Design review of the part built by this model. Coordinates are the model's own, in mm. Face numbers are marked on the shaded views. A direction names the side the tool comes from. Give positions to 0.01 mm unless a question says otherwise; leave off trailing zeros. Order: outer loops, then holes, each group sorted by start corner. A loop starts at its lowest first (then second) coordinate and runs counter-clockwise, first axis right, second up. Notation, with made-up numbers: (14, 11) - (48, 11) arc R22 ccw to (48, 32) - close; hole circle Ø10 at (52.25, 68). An arc over 180 degrees is marked (long way). Write each question's results on one line, items separated by ' | '. Start each with the question number.
```python
from build123d import *

# Parameters (mm, degrees)
SKETCH1_W           = 100
SKETCH1_H           = 20
BOSS_EXTRUDE1_DEPTH = 8
FILLET1_R           = 5
SKETCH2_R           = 29.154376269
BOSS_EXTRUDE3_DEPTH = 20
SKETCH3_R           = 2.9
CUT_EXTRUDE1_DEPTH  = 26
SKETCH4_R           = 21
CUT_EXTRUDE2_DEPTH  = 74


with BuildPart() as part:
    # Sketch1 → Boss-Extrude1 (new body)
    with BuildSketch(Plane(origin=(0, 0, 0), x_dir=(1, 0, 0), z_dir=(0, 1, 0))):
        Rectangle(SKETCH1_W, SKETCH1_H)
    extrude(amount=BOSS_EXTRUDE1_DEPTH)

    # Fillet1
    fillet1_edges = [part.edges().sort_by_distance(p)[0] for p in [
        (-50, 8, 0),
        (50, 8, 0),
    ]]
    fillet(fillet1_edges, radius=FILLET1_R)

    # Sketch2 → Boss-Extrude3 (add)
    with BuildSketch(Plane.XY.offset(10)):
        with Locations((0, 31.226436769)):
            Circle(SKETCH2_R)
    extrude(amount=-BOSS_EXTRUDE3_DEPTH)

    # Sketch3 → Cut-Extrude1 (cut)
    with BuildSketch(Plane(origin=(0, 8, 0), x_dir=(1, 0, 0), z_dir=(0, 1, 0))):
        with Locations(Location((-36.246581996, 0, 0), (0, 0, 270))):
            Circle(SKETCH3_R)
        with Locations(Location((36.246581996, 0, 0), (0, 0, 270))):
            Circle(SKETCH3_R)
    extrude(amount=-CUT_EXTRUDE1_DEPTH, mode=Mode.SUBTRACT)

    # Sketch4 → Cut-Extrude2 (cut)
    with BuildSketch(Plane.XY.offset(10)):
        with Locations((0, 31.226436769)):
            Circle(SKETCH4_R)
    extrude(amount=-CUT_EXTRUDE2_DEPTH, mode=Mode.SUBTRACT)


solid = part.part
```
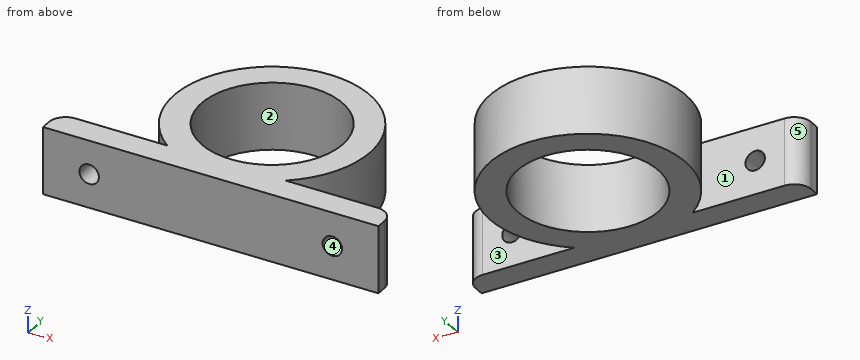
Q1. Draft analysis for pull direction Y (two halves, no side actions). For the marked faces 3, 4 and 5, state which applies: pulls with the +Y half, pulls with the -Y half, needs draft (parallel to the pull), parting line crosses it, or undercut.
Q2. Add section A-A (x = 0). Give the boundary of the cut face in (y, z).
Q3. Insertion check: pin 1 Ø3 at (y, z) = (6.5, -4) entering from -X; pin 2 Ø10 at (y, z) = (28, 7) entering from -X; pin 3 Ø25 at (x, y) = (0, 31.23) entering from -Z; pin 4 Ø10 at (y, z) = (42.5, 7.5) entering from -X. Each pin has a flat end and moves straight along its axis. Give the tip position at first contact, or say it passes through.
Q4. Add section B-B (z = -0.5). Give the boundary of the cut face in (x, y), plus the area to 3 significant figures.
Q5. Machinability: for the marked faces 1 and 2, which of the approach directions +Z, -Z, +X, -X, +Y, -Y give a long, thin tool a straight path to every point of the face, cutting with its end or side? Answer none if there is none.
Q6. Add section D-D (z = 8). Give the boundary of the cut face in (x, y).
Q7. Add section C-C (y = 25.5). Give the boundary of the cut face in (x, z), plus the area to 3 significant figures.
Q8. For line 1 (X direction, y = 4.5, z = 0); line 2 (X direction, y = 3.5, z = 1.5); line 3 (Y direction, x = 1, z = -3.25), list the stretches that pass through material, from the lowest coordinate up. Write a range as [from, to].
Verdict:
1) face 3: undercut | face 4: needs draft | face 5: pulls with the +Y half
2) outline: (0, -10) - (10.23, -10) - (10.23, 10) - (0, 10) - close; (52.23, -10) - (60.38, -10) - (60.38, 10) - (52.23, 10) - close
3) pin 1: stops at x = -49.58 | pin 2: stops at x = -29.15 | pin 3: passes through | pin 4: stops at x = -28.47
4) outline: (-50, 0) - (-39.1, 0) - (-39.1, 8) - (-45, 8) arc R5 ccw to (-50, 3) - close; (-33.39, 0) - (33.39, 0) - (33.39, 8) - (17.62, 8) arc R29.15 ccw (long way) to (-17.62, 8) - (-33.39, 8) - close; (39.1, 0) - (50, 0) - (50, 3) arc R5 ccw to (45, 8) - (39.1, 8) - close; hole circle Ø42 at (0, 31.23) | area: 1,840 mm2
5) face 1: +Z, -Z, -X | face 2: +Z, -Z
6) outline: (-50, 0) - (50, 0) - (50, 3) arc R5 ccw to (45, 8) - (17.62, 8) arc R29.15 ccw (long way) to (-17.62, 8) - (-45, 8) arc R5 ccw to (-50, 3) - close; hole circle Ø42 at (0, 31.23)
7) outline: (-28.59, -10) - (-20.2, -10) - (-20.2, 10) - (-28.59, 10) - close; (20.2, -10) - (28.59, -10) - (28.59, 10) - (20.2, 10) - close | area: 335 mm2
8) line 1: x = [-49.77, -39.15], [-33.35, 33.35], [39.15, 49.77] | line 2: x = [-49.97, -38.73], [-33.76, 33.76], [38.73, 49.97] | line 3: y = [0, 10.25], [52.2, 60.36]
